Could you check a few things on this drawing? It's one solid part, dimensions in mm from its lowest x, y, z. Give positions to 0.01 mm unless a question says otherwise; leave off trailing zeros. Write each loop counter-clockwise with the first axis right and the second up, starting at its lowest first coordinate (ties: lowest second). Pieces come first, ordered by that corner, then holes.
1. I'm going to push a flat-ended pin straight in: pin 1 (6 mm diameter, centred on y = 6.5, z = 59.5, fed in from -X). Where does the tip first touch, or does it pass through?
2. Suppose I cut it at A-A (z = 60). Please give me the cut outline in (x, y), and give its area (3 significant figures).
3. Suppose I cut it at C-C (z = 7.5). Please give me the cut outline in (x, y).
4. Suppose I cut it at D-D (y = 13.5). Please give me the cut outline in (x, z).
5. If I drill on probe 1 along X at (y, z) = (2.5, 55); probe 2 along Z at (x, y) = (94, 16); probe 3 along Z at (x, y) = (96, 23), over which ranges is the centre line in solid material (lowest first)?
6. Suppose I cut it at B-B (x = 36). Please give me the cut outline in (y, z), and give its area (3 significant figures).
7. Thinking about a two-plate mould opening in X: for the marked faces 1, 2, 3 and 4, which applies, pulls with the +X half, pulls with the -X half, needs draft (parallel to the pull), parting line crosses it, or undercut?
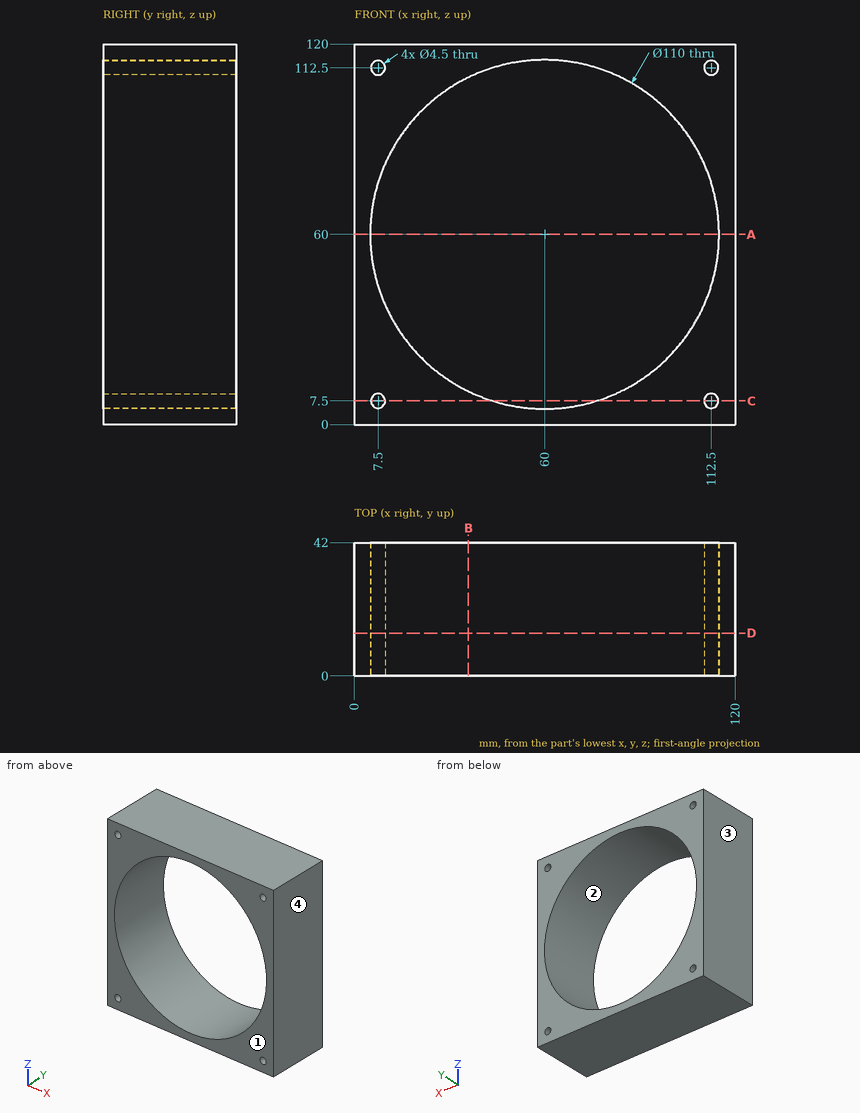
Checks:
1. pin 1: stops at x = 0
2. outline: (0, 0) - (5, 0) - (5, 42) - (0, 42) - close; (115, 0) - (120, 0) - (120, 42) - (115, 42) - close
2. area: 420 mm2
3. outline: (0, 0) - (5.25, 0) - (5.25, 42) - (0, 42) - close; (9.75, 0) - (43.61, 0) - (43.61, 42) - (9.75, 42) - close; (76.39, 0) - (110.25, 0) - (110.25, 42) - (76.39, 42) - close; (114.75, 0) - (120, 0) - (120, 42) - (114.75, 42) - close
4. outline: (0, 0) - (120, 0) - (120, 120) - (0, 120) - close; hole circle Ø110 at (60, 60); hole circle Ø4.5 at (7.5, 7.5); hole circle Ø4.5 at (7.5, 112.5); hole circle Ø4.5 at (112.5, 7.5); hole circle Ø4.5 at (112.5, 112.5)
5. probe 1: x = 0 to 5.23, 114.77 to 120
5. probe 2: z = 0 to 16.77, 103.23 to 120
5. probe 3: z = 0 to 18.42, 101.58 to 120
6. outline: (0, 0) - (42, 0) - (42, 10.51) - (0, 10.51) - close; (0, 109.49) - (42, 109.49) - (42, 120) - (0, 120) - close
6. area: 883 mm2
7. face 1: needs draft
7. face 2: undercut
7. face 3: pulls with the -X half
7. face 4: pulls with the +X half
